from build123d import *

# Parameters (mm, degrees)
SKETCH1_W           = 480
SKETCH1_H           = 650
BOSS_EXTRUDE1_DEPTH = 10
FILLET2_R           = 60
SKETCH3_W           = 130
SKETCH3_H           = 150
CUT_EXTRUDE1_DEPTH  = 10
SKETCH5_W           = 562.756234426
SKETCH5_H           = 100
CUT_EXTRUDE2_DEPTH  = 10
FILLET3_R           = 10


with BuildPart() as part:
    # Sketch1 → Boss-Extrude1 (new body)
    with BuildSketch(Plane(origin=(0, 0, 0), x_dir=(1, 0, 0), z_dir=(0, 1, 0))):
        Rectangle(SKETCH1_W, SKETCH1_H)
    extrude(amount=BOSS_EXTRUDE1_DEPTH)

    # Fillet2
    fillet2_edges = [part.edges().sort_by_distance(p)[0] for p in [
        (240, 5, 325),
        (-240, 5, 325),
        (-240, 5, -325),
        (240, 5, -325),
    ]]
    fillet(fillet2_edges, radius=FILLET2_R)

    # Sketch3 → Cut-Extrude1 (cut)
    with BuildSketch(Plane(origin=(0, 10, 0), x_dir=(1, 0, 0), z_dir=(0, 1, 0))):
        with Locations((240, 0)):
            Rectangle(SKETCH3_W, SKETCH3_H)
        with Locations((-240, 0)):
            Rectangle(SKETCH3_W, SKETCH3_H)
    extrude(amount=-CUT_EXTRUDE1_DEPTH, mode=Mode.SUBTRACT)

    # Sketch5 → Cut-Extrude2 (cut)
    with BuildSketch(Plane(origin=(0, 10, 0), x_dir=(1, 0, 0), z_dir=(0, 1, 0))):
        with Locations((0, -275)):
            Rectangle(SKETCH5_W, SKETCH5_H)
        with Locations((0, 275)):
            Rectangle(SKETCH5_W, SKETCH5_H)
    extrude(amount=-CUT_EXTRUDE2_DEPTH, mode=Mode.SUBTRACT)

    # Fillet3
    fillet3_edges = [part.edges().sort_by_distance(p)[0] for p in [
        (-240, 5, 75),
        (-175, 5, 75),
        (-240, 5, -75),
        (-175, 5, -75),
        (240, 5, -75),
        (175, 5, -75),
        (240, 5, 75),
        (175, 5, 75),
        (-240, 5, 225),
        (240, 5, -225),
        (240, 5, 225),
        (-240, 5, -225),
    ]]
    fillet(fillet3_edges, radius=FILLET3_R)


solid = part.part
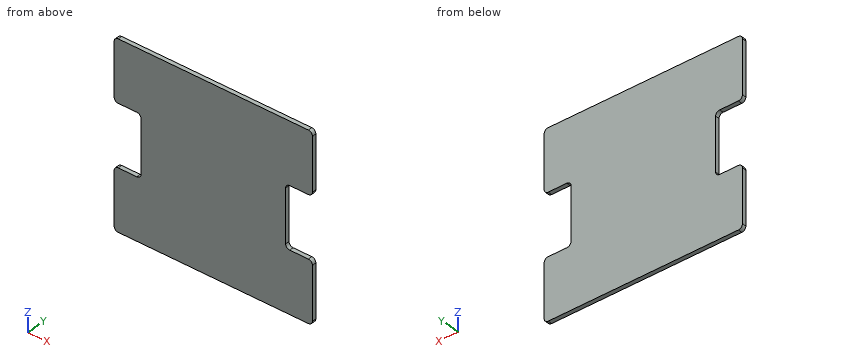
The model under review builds one solid part; all positions refer to its coordinate system, in mm. Give positions to 0.01 mm unless a question says otherwise; leave off trailing zeros. Loops run counter-clockwise (first coordinate to the right, second up) from the corner with the lowest first, then second, coordinate; pieces in that order, holes last. Notation, with made-up numbers: (8.25, 60.5) -> (32.25, 60.5) arc R26 ccw to (32.25, 87.5) -> close; hole circle Ø4 at (13.25, -3). An arc over 180 degrees is marked (long way). Put each result on its own line as item: value. Start each with the question number.
1. Clearance check with flat-ended pins moving along their axes: P1, Ø3, axis at y = 4, z = -5, coming from the +X side; P2, Ø5, axis at y = 5, z = -5.5, coming from the -X side. State where each tip first meets the part, or that it passes through.
2. We need section B-B on z = -6.5. State the section outline as (x, y) points.
3. Wall thickness on probe 1 along Z at (x, y) = (-213, 5.75); probe 2 along X at (y, z) = (7.75, 8); probe 3 along Z at (x, y) = (184, 7.5): over which ranges is each line inside the solid? List them lowest first.
4. We need section A-A on y = 2.75. State the section outline as (x, z) points, then the cut area to 3 significant figures.
Determined:
1. P1: x = 175
1. P2: x = -175
2. outline: (-175, 0) -> (175, 0) -> (175, 10) -> (-175, 10) -> close
3. probe 1: -225 to -75, 75 to 225
3. probe 2: -175 to 175
3. probe 3: -225 to -74.95, 74.95 to 225
4. outline: (-240, -215) arc R10 ccw to (-230, -225) -> (230, -225) arc R10 ccw to (240, -215) -> (240, -85) arc R10 ccw to (230, -75) -> (185, -75) arc R10 cw to (175, -65) -> (175, 65) arc R10 cw to (185, 75) -> (230, 75) arc R10 ccw to (240, 85) -> (240, 215) arc R10 ccw to (230, 225) -> (-230, 225) arc R10 ccw to (-240, 215) -> (-240, 85) arc R10 ccw to (-230, 75) -> (-185, 75) arc R10 cw to (-175, 65) -> (-175, -65) arc R10 cw to (-185, -75) -> (-230, -75) arc R10 ccw to (-240, -85) -> close
4. area: 196,000 mm^2
